```python
from build123d import *

# Parameters (mm, degrees)
BASE_BLOCK_DEPTH                = 58
FRONT_BORE_BOSS_DEPTH           = 58
FRONT_BORE_SKETCH_R             = 7
FRONT_BORE_DEPTH                = 73.698005475
LEFT_ARM_SKETCH_R               = 8
LEFT_ARM_SKETCH_R_2             = 4
LEFT_ARM_DEPTH                  = 5
LEFT_ARM_WEB_DEPTH              = 5
LEFT_START                      = 5
LEFT_PIVOT_BOSS_SKETCH_R        = 8
LEFT_PIVOT_BOSS_DEPTH           = 5
LEFT_PIVOT_HOLE_SKETCH_R        = 4
LEFT_PIVOT_HOLE_DEPTH           = 85.711274338
RIGHT_ARM_SKETCH_R              = 8
RIGHT_ARM_SKETCH_R_2            = 4
RIGHT_ARM_DEPTH                 = 5
RIGHT_ARM_WEB_DEPTH             = 5
RIGHT_PIVOT_BOSS_SKETCH_R       = 8
RIGHT_PIVOT_BOSS_DEPTH          = 5
RIGHT_PIVOT_HOLE_8_SKETCH_R     = 4
RIGHT_PIVOT_HOLE_8_DEPTH        = 87.377080293
SIDE_LUG_SKETCH_R               = 4
SIDE_LUG_DEPTH                  = 5
MOUNTING_TAB_SKETCH_W           = 16
MOUNTING_TAB_SKETCH_H           = 58
MOUNTING_TAB_DEPTH              = 5
M5_COUNTERBORE_HOLE_D           = 4.5
M5_COUNTERBORE_HOLE_CBORE_D     = 9.53
M5_COUNTERBORE_HOLE_CBORE_DEPTH = 2.67


with BuildPart() as part:
    # Base Block Profile → Base Block (new body)
    with BuildSketch(Plane.XY):
        Polygon((0, 0), (6, 0), (6, 2), (30, 2), (30, 0), (36, 0), (36, 22), (0, 22), align=None)
    extrude(amount=BASE_BLOCK_DEPTH)

    # Front Bore Boss Sketch → Front Bore Boss (add, through all)
    with BuildSketch(Plane.XY.offset(58)):
        with BuildLine():
            Line((4, 11), (32, 11))
            ThreePointArc((32, 11), (18, 25), (4, 11))
        make_face()
    extrude(amount=-FRONT_BORE_BOSS_DEPTH)

    # Front Bore Sketch → Front Bore (cut, through all)
    with BuildSketch(Plane.XY.offset(58)):
        with Locations((18, 11)):
            Circle(FRONT_BORE_SKETCH_R)
    extrude(amount=-FRONT_BORE_DEPTH, mode=Mode.SUBTRACT)



with BuildPart() as body_2:
    # Left Arm Sketch → Left Arm (new, symmetric)
    with BuildSketch(Plane(origin=(0, 0, 0), x_dir=(0, 0, -1), z_dir=(1, 0, 0))):
        with Locations((-29, 48)):
            Circle(LEFT_ARM_SKETCH_R)
        with Locations((-29, 48)):
            Circle(LEFT_ARM_SKETCH_R_2, mode=Mode.SUBTRACT)
    extrude(amount=LEFT_ARM_DEPTH, both=True)


with BuildPart() as part_1:
    add(part.part)

    add(body_2.part)  # Left Arm Web merges body 2
    # Left Arm Web Sketch → Left Arm Web (add)
    with BuildSketch(Plane(origin=(0, 0, 0), x_dir=(0, 0, -1), z_dir=(1, 0, 0))):
        with BuildLine():
            Line((-21, 48), (0, 22))
            Line((0, 22), (-58, 22))
            Line((-58, 22), (-37, 48))
            ThreePointArc((-37, 48), (-29, 40), (-21, 48))
        make_face()
    extrude(amount=LEFT_ARM_WEB_DEPTH)

    # Left Pivot Boss Sketch → Left Pivot Boss (add)
    with BuildSketch(Plane(origin=(5, 0, 0), x_dir=(0, 0, -1), z_dir=(1, 0, 0)).offset(LEFT_START)):
        with Locations((-29, 48)):
            Circle(LEFT_PIVOT_BOSS_SKETCH_R)
    extrude(amount=-LEFT_PIVOT_BOSS_DEPTH)

    # Left Pivot Hole Sketch → Left Pivot Hole (cut, through all)
    with BuildSketch(Plane(origin=(10, 0, 0), x_dir=(0, 0, -1), z_dir=(1, 0, 0))):
        with Locations((-29, 48)):
            Circle(LEFT_PIVOT_HOLE_SKETCH_R)
    extrude(amount=-LEFT_PIVOT_HOLE_DEPTH, mode=Mode.SUBTRACT)



with BuildPart() as body_2_2:
    # Right Arm Sketch → Right Arm (new, symmetric)
    with BuildSketch(Plane(origin=(36, 0, 0), x_dir=(0, 0, -1), z_dir=(1, 0, 0))):
        with Locations((-29, 48)):
            Circle(RIGHT_ARM_SKETCH_R)
        with Locations((-29, 48)):
            Circle(RIGHT_ARM_SKETCH_R_2, mode=Mode.SUBTRACT)
    extrude(amount=RIGHT_ARM_DEPTH, both=True)


with BuildPart() as part_2:
    add(part_1.part)

    add(body_2_2.part)  # Right Arm Web merges body 2 2
    # Right Arm Web Sketch → Right Arm Web (add)
    with BuildSketch(Plane(origin=(36, 0, 0), x_dir=(0, 0, -1), z_dir=(1, 0, 0))):
        with BuildLine():
            Line((-37, 48), (-58, 22))
            Line((-58, 22), (0, 22))
            Line((0, 22), (-21, 48))
            ThreePointArc((-21, 48), (-29, 40), (-37, 48))
        make_face()
    extrude(amount=-RIGHT_ARM_WEB_DEPTH)

    # Right Pivot Boss Sketch → Right Pivot Boss (add)
    with BuildSketch(Plane.ZY.offset(-31)):
        with Locations(Location((29, 48, 0), (0, 0, 180))):
            Circle(RIGHT_PIVOT_BOSS_SKETCH_R)
    extrude(amount=RIGHT_PIVOT_BOSS_DEPTH)

    # Right Pivot Hole Ø8 Sketch → Right Pivot Hole Ø8 (cut, through all)
    with BuildSketch(Plane.ZY.offset(-26)):
        with Locations(Location((29, 48, 0), (0, 0, 180))):
            Circle(RIGHT_PIVOT_HOLE_8_SKETCH_R)
    extrude(amount=-RIGHT_PIVOT_HOLE_8_DEPTH, mode=Mode.SUBTRACT)

    # Side Lug Sketch → Side Lug (add)
    with BuildSketch(Plane(origin=(0, 0, 0), x_dir=(1, 0, 0), z_dir=(0, 1, 0))):
        with BuildLine():
            Line((52, -21), (36, -21))
            Line((36, -21), (36, -37))
            Line((36, -37), (52, -37))
            ThreePointArc((52, -37), (60, -29), (52, -21))
        make_face()
        with Locations(Location((52, -29, 0), (0, 0, 270))):
            Circle(SIDE_LUG_SKETCH_R, mode=Mode.SUBTRACT)
    extrude(amount=SIDE_LUG_DEPTH)

    # Mounting Tab Sketch → Mounting Tab (add)
    with BuildSketch(Plane(origin=(0, 0, 0), x_dir=(1, 0, 0), z_dir=(0, 1, 0))):
        with Locations((-8, -29)):
            Rectangle(MOUNTING_TAB_SKETCH_W, MOUNTING_TAB_SKETCH_H)
    extrude(amount=MOUNTING_TAB_DEPTH)

    # M5 Counterbore Hole (through all)
    with Locations(Plane(origin=(0, 5, 0), x_dir=(1, 0, 0), z_dir=(0, 1, 0))):
        with Locations((-8, -8), (-8, -50)):
            CounterBoreHole(M5_COUNTERBORE_HOLE_D / 2, M5_COUNTERBORE_HOLE_CBORE_D / 2, M5_COUNTERBORE_HOLE_CBORE_DEPTH)


solid = part_2.part
```
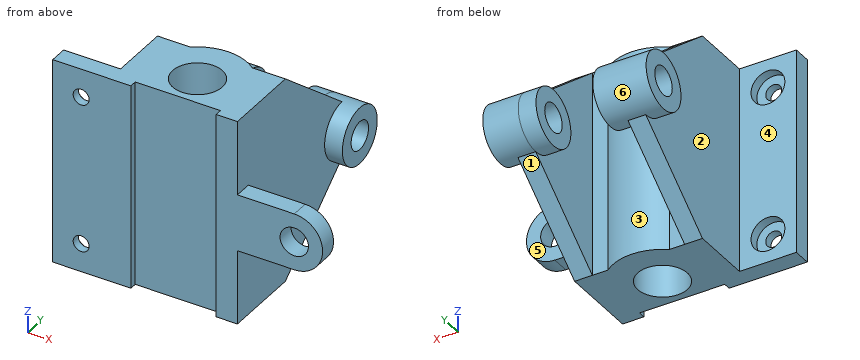
Could you check a few things on this model? Use its own coordinates, in mm. Face numbers are marked on the shaded views. A direction names the side the tool comes from. Coordinates: 2 decimals unless noted, no trailing zeros. Order: outer loops, then holes, each group sorted by start corner. A loop starts at its lowest first (then second) coordinate and runs counter-clockwise, first axis right, second up. Notation, with made-up numbers: M 28,48.5 L 67,48.5 A17 ccw 67,58.5 Z; hole C 61.25,51.5 d9. An arc over 180 degrees is marked long. Use a Markdown table: item, result. Add a question column.
Q1. I want a section at D-D on z = 8. List the corners of the cut face in (x, y) for me (3 decimals), then the cut area to 3 significant figures.
Q2. Which directions (+Z, -Z, +X, -X, +Y, -Y) give clear straight access to the entire face, cutting with the end or side of a thin tool? Please do the marked faces 4, 5 and 6.
Q3. I want a section at B-B on x = -8. List the corners of the cut face in (y, z) for me (3 decimals).
Q4. We'd pull the mould along X, two halves only. Please class the marked faces 1, 2 and 3: pulls with the +X half, pulls with the -X half, needs draft (parallel to the pull), parting line crosses it, or undercut.
Q5. If I drill on L1, parallel to Z at x = -8, y = 3.15 (3 decimals); L2, parallel to Y at x = 27.95, z = 29; L3, parallel to X at y = 38, z = 39.5, over which ranges is the centre line in solid material (lowest first)?
Q6. I want a section at C-C on x = 18. List the corners of the cut face in (y, z) for me, then the cut area to 3 significant figures.
Q7. I'm going to push flat-ended pins straight in: pin 1 (1.5 mm diameter, centred on x = 42.5, y = 3.5, fed in from +Z); pin 2 (5 mm diameter, centred on x = 46, z = 31, fed in from -Y); pin 3 (2 mm diameter, centred on y = 11.5, z = 15, fed in from -X); pin 4 (13 mm diameter, centred on y = 51, z = 28, fed in from -X). Where does each tip first touch, or does it pass through?
Q8. I want a section at A-A on y = 11. List the corners of the cut face in (x, z) for me.
Checked values:
| question | item | result |
|---|---|---|
| 1 | outline | M -16,0 L -10.25,0 L -10.25,2.33 L -12.765,2.33 L -12.765,5 L -16,5 Z; M -5.75,0 L 6,0 L 6,2 L 30,2 L 30,0 L 36,0 L 36,31.905 L 31,31.905 L 31,22 L 26.66,22 A14 ccw 9.34,22 L 5,22 L 5,31.905 L 0,31.905 L 0,5 L -3.235,5 L -3.235,2.33 L -5.75,2.33 Z; hole C 18,11 d14 |
| 1 | area | 769 mm² |
| 2 | face 4 | +Z, -Z, -X |
| 2 | face 5 | +Z, -Z, +X |
| 2 | face 6 | none |
| 3 | outline | M 0,0 L 5,0 L 5,3.235 L 2.33,3.235 L 2.33,5.75 L 0,5.75 Z; M 0,10.25 L 2.33,10.25 L 2.33,12.765 L 5,12.765 L 5,45.235 L 2.33,45.235 L 2.33,47.75 L 0,47.75 Z; M 0,52.25 L 2.33,52.25 L 2.33,54.765 L 5,54.765 L 5,58 L 0,58 Z |
| 4 | face 1 | needs draft |
| 4 | face 2 | pulls with the -X half |
| 4 | face 3 | undercut |
| 5 | L1 | 0 to 3.235, 12.765 to 45.235, 54.765 to 58 |
| 5 | L2 | 2 to 22, 40 to 44, 52 to 56 |
| 5 | L3 | 0 to 5, 31 to 36 |
| 6 | outline | M 2,0 L 4,0 L 4,58 L 2,58 Z; M 18,0 L 25,0 L 25,58 L 18,58 Z |
| 6 | area | 522 mm² |
| 7 | pin 1 | z = 37 |
| 7 | pin 2 | y = 0 |
| 7 | pin 3 | x = 0 |
| 7 | pin 4 | x = -5 |
| 8 | outline | M 0,0 L 11,0 L 11,58 L 0,58 Z; M 25,0 L 36,0 L 36,58 L 25,58 Z |
